Geometry: final body of the model. Coordinates: model frame, mm. A direction names the side the tool comes from. Coordinates: 2 decimals unless noted, no trailing zeros. Write each loop counter-clockwise with the first axis right and the second up, starting at its lowest first coordinate (ties: lowest second). Pieces come first, ordered by that corner, then holes. Notation, with made-up numbers: (22.5, -1) - (63.5, -1) arc R21 cw to (63.5, 27) - close; hole circle Ø10 at (-27.5, 44.5). An arc over 180 degrees is marked (long way). Answer as a JSON object with one key per item and string values. Group by question number.
Item 1: Section A-A on y = 0. State how many separate pieces and enclosed holes the cut face has, and give its area (3 significant figures).
Item 2: Set-up query: faces 5 (the cylindrical face through (-23.89, 1.35, -2.1)), 6 (the cylindrical face through (-44.505, 0.242, -0.648)). Return all of +Z, -Z, +X, -X, +Y, -Y with unobstructed straight access to the full face (end or side cutting, diameter ignored); none if empty.
Item 3: First-contact query: pin 1 Ø9 at (x, y) = (51, -1) entering from -Z; pin 2 Ø10.5 at (x, y) = (50, 0) entering from -Z; pin 3 Ø14.5 at (x, y) = (20.4, 0) entering from +Z. Flat tips, straight axial feed; report the tip coordinate or a pass-through.
Item 4: Mould query, pull axis X, two halves, no side actions, for faces 1 (the flat face through (-60, 0, 1)), 2 (the flat face through (-1, -20, 1)), 3 (the flat face through (-54, 0, 2.8)), 4 (the flat face through (60, 0, 1)). Classes: pulls with the +X half, pulls with the -X half, needs draft (parallel to the pull), parting line crosses it, or undercut.
Item 5: Section B-B on x = -50. Return loops of the section in (y, z).
Item 6: Line query: line 1 along X through (y, z) = (2, -3.25); line 2 along Y through (x, z) = (-50, 3.4); line 3 along X through (y, z) = (3.5, -1.5). Output: solid intervals per line, ascending. Write a range as from..to.
Item 7: Section C-C on z = 1. Return loops of the section in (x, y), and give its area (3 significant figures).
```python
from build123d import *

# Parameters (mm, degrees)
SKETCH_1_W                  = 120
SKETCH_1_H                  = 40
EXTRUDE_1_DEPTH             = 4
HOLE_WIZARD_1_D             = 9
HOLE_WIZARD_1_DEPTH         = 10
HOLE_WIZARD_1_CSINK_D       = 17.3
HOLE_WIZARD_1_CSINK_ANGLE   = 90
HOLE_WIZARD_1_TIP           = 2.703872786
HOLE_WIZARD_1_2_D           = 6.6
HOLE_WIZARD_1_2_DEPTH       = 10
HOLE_WIZARD_1_2_CBORE_D     = 11
HOLE_WIZARD_1_2_CBORE_DEPTH = 6.8
HOLE_WIZARD_1_2_TIP         = 1.982840043
CHAMFER_1_SIZE              = 1


with BuildPart() as part:
    # 草图1 → 凸台-拉伸1 (new, symmetric)
    with BuildSketch(Plane.XY):
        Rectangle(SKETCH_1_W, SKETCH_1_H)
    extrude(amount=EXTRUDE_1_DEPTH, both=True)

    # Hole Wizard 1
    with Locations(Plane(origin=(-19.595917942, 0, 4), x_dir=(1, 0, 0), z_dir=(0, 0, 1))):
        with Locations((0, 0), (40, 0)):
            CounterSinkHole(HOLE_WIZARD_1_D / 2, HOLE_WIZARD_1_CSINK_D / 2, depth=HOLE_WIZARD_1_DEPTH, counter_sink_angle=HOLE_WIZARD_1_CSINK_ANGLE)
            with Locations((0, 0, -(HOLE_WIZARD_1_DEPTH + HOLE_WIZARD_1_TIP / 2))):  # 118° drill point
                Cone(0, HOLE_WIZARD_1_D / 2, HOLE_WIZARD_1_TIP, mode=Mode.SUBTRACT)

    # Hole Wizard 1 2
    with Locations(Plane(origin=(50, 0, -4), x_dir=(-1, 0, 0), z_dir=(0, 0, -1))):
        with Locations((0, 0), (100, 0)):
            CounterBoreHole(HOLE_WIZARD_1_2_D / 2, HOLE_WIZARD_1_2_CBORE_D / 2, HOLE_WIZARD_1_2_CBORE_DEPTH, depth=HOLE_WIZARD_1_2_DEPTH)
            with Locations((0, 0, -(HOLE_WIZARD_1_2_DEPTH + HOLE_WIZARD_1_2_TIP / 2))):  # 118° drill point
                Cone(0, HOLE_WIZARD_1_2_D / 2, HOLE_WIZARD_1_2_TIP, mode=Mode.SUBTRACT)

    # 倒角1
    chamfer_1_edges = [part.edges().sort_by_distance(p)[0] for p in [
        (0, -20, -4),
        (-60, 0, -4),
        (0, 20, -4),
        (60, 0, -4),
    ]]
    chamfer(chamfer_1_edges, length=CHAMFER_1_SIZE)


solid = part.part
```
Checks:
{
 "1": {"separate pieces": "5", "enclosed holes": "0", "area": "615 mm^2"},
 "2": {"face 5": "+Z, -Z", "face 6": "-Z"},
 "3": {"pin 1": "z = -4", "pin 2": "z = 2.8", "pin 3": "z = 2.6"},
 "4": {"face 1": "pulls with the -X half", "face 2": "needs draft", "face 3": "undercut", "face 4": "pulls with the +X half"},
 "5": {"outline": "(-20, -3) - (-19, -4) - (-5.5, -4) - (-5.5, 2.8) - (-3.3, 2.8) - (-3.3, 4) - (-20, 4) - close; (3.3, 2.8) - (5.5, 2.8) - (5.5, -4) - (19, -4) - (20, -3) - (20, 4) - (3.3, 4) - close"},
 "6": {"line 1": "-59.75..-55.12, -44.88..-23.63, -15.56..16.37, 24.44..44.88, 55.12..59.75", "line 2": "-20..-3.3, 3.3..20", "line 3": "-60..-54.24, -45.76..-22.42, -16.77..17.58, 23.23..45.76, 54.24..60"},
 "7": {"outline": "(-60, -20) - (60, -20) - (60, 20) - (-60, 20) - close; hole circle Ø11 at (-50, 0); hole circle Ø11.3 at (-19.6, 0); hole circle Ø11.3 at (20.4, 0); hole circle Ø11 at (50, 0)", "area": "4,410 mm^2"}
}
